The model under review builds one solid part; all positions refer to its coordinate system, in mm. Give positions to 0.01 mm unless a question says otherwise; leave off trailing zeros. Loops run counter-clockwise (first coordinate to the right, second up) from the corner with the lowest first, then second, coordinate; pieces in that order, holes last. Notation, with made-up numbers: (46, 14) -> (58, 14) arc R16 cw to (58, 35) -> close; hole circle Ø6 at (-0.75, 1.25). An arc over 180 degrees is marked (long way). Write each question's results on one line, items separated by ' | '. Start each with the question number.
Q1. Wall thickness on L1, parallel to Y at x = 1534.5, z = 1.5; L2, parallel to Y at x = 930.5, z = 0: over which ranges is each line inside the solid? List them lowest first. Write a range as [from, to].
Q2. We need section B-B (y = -706). Write out the cut boundary in (x, z), plus the area to 3 significant figures.
Q3. We need section A-A (z = 0). Write out the cut boundary in (x, y).
Q4. Insertion check: pin 1 Ø4 at (y, z) = (-473.5, 7) entering from -X; pin 2 Ø6 at (y, z) = (-815.5, -7.5) entering from -X; pin 3 Ø12 at (x, z) = (1008, -1) entering from -Y. Each pin has a flat end and moves straight along its axis. Give the tip position at first contact, or say it passes through.
from build123d import *

# Parameters (mm, degrees)
SWEEP_THIN1_PROFILE_R   = 10
SWEEP_THIN1_PROFILE_R_2 = 8


with BuildPart() as part:
    # Sweep-Thin1: sweep along a path in Sketch1
    with BuildLine(Plane.XY) as sweep_thin1_path:
        Line((2300, 0), (60, 0))
        ThreePointArc((60, 0), (17.573593129, -17.573593129), (0, -60))
        Line((0, -60), (0, -1000))
    # Sweep-Thin1 profile (on start of the path) → Sweep-Thin1 (sweep)
    with BuildSketch(Plane(origin=(2300, 0, 0), x_dir=(0, 0, -1), z_dir=(-1, 0, 0))):
        Circle(SWEEP_THIN1_PROFILE_R)
        Circle(SWEEP_THIN1_PROFILE_R_2, mode=Mode.SUBTRACT)
    sweep(path=sweep_thin1_path.line)


solid = part.part
Output:
1) L1: [-9.89, -7.86], [7.86, 9.89] | L2: [-10, -8], [8, 10]
2) outline: circle Ø20 at (0, 0); hole circle Ø16 at (0, 0) | area: 113 mm2
3) outline: (-10, -1000) -> (-8, -1000) -> (-8, -60) arc R68 cw to (60, 8) -> (2300, 8) -> (2300, 10) -> (60, 10) arc R70 ccw to (-10, -60) -> close; (8, -1000) -> (10, -1000) -> (10, -60) arc R50 cw to (60, -10) -> (2300, -10) -> (2300, -8) -> (60, -8) arc R52 ccw to (8, -60) -> close
4) pin 1: x = -8.66 | pin 2: x = -8.93 | pin 3: y = -10
